Could you check a few things on this model? Use its own coordinates, in mm. Coordinates: 2 decimals unless noted, no trailing zeros. Loops run counter-clockwise (first coordinate to the right, second up) from the corner with the lowest first, then second, coordinate; pieces in that order, holes last. Notation, with made-up numbers: (-10.5, 88) - (30.5, 88) arc R25 cw to (30.5, 117) - close; hole circle Ø3 at (44.25, -32.75). An arc over 180 degrees is marked (long way). Use CSV: the item, a comma, the result in double quotes.
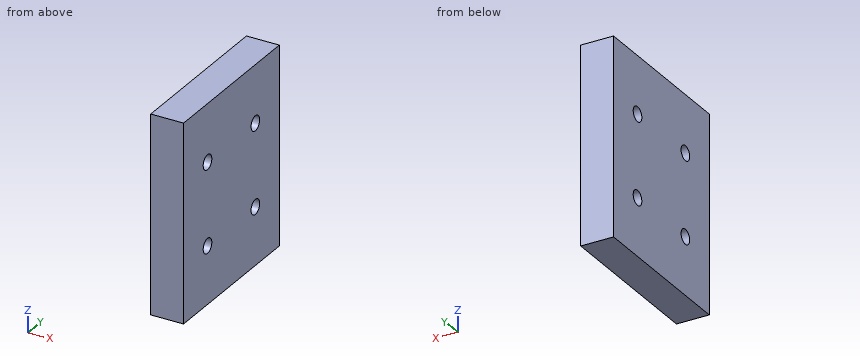
from build123d import *

# Parameters (mm, degrees)
SKETCH_1_W            = 120
SKETCH_1_H            = 100
EXTRUDE_1_DEPTH       = 20
HOLE_WIZARD_9_0_9_1_D = 9


with BuildPart() as part:
    # 草图1 → 凸台-拉伸1 (new body)
    with BuildSketch(Plane(origin=(0, 0, 0), x_dir=(0, 0, -1), z_dir=(1, 0, 0))):
        Rectangle(SKETCH_1_W, SKETCH_1_H)
    extrude(amount=EXTRUDE_1_DEPTH)

    # Ø9.0 (9) 直径孔1 (through all)
    with Locations(Plane(origin=(20, 0, 0), x_dir=(0, 0, -1), z_dir=(1, 0, 0))):
        with Locations((-25, 25), (25, 25), (-25, -25), (25, -25)):
            Hole(HOLE_WIZARD_9_0_9_1_D / 2)


solid = part.part
(1) Suppose I cut it at B-B (z = 25). Write out the boundary of the cut face in (x, y).
Computed:
outline,"(0, -50) - (20, -50) - (20, -29.5) - (0, -29.5) - close; (0, -20.5) - (20, -20.5) - (20, 20.5) - (0, 20.5) - close; (0, 29.5) - (20, 29.5) - (20, 50) - (0, 50) - close"
(2) Suppose I cut it at A-A (x = 11.25). Write out the boundary of the cut face in (y, z), plus the area to 3 significant figures.
Computed:
outline,"(-50, -60) - (50, -60) - (50, 60) - (-50, 60) - close; hole circle Ø9 at (-25, -25); hole circle Ø9 at (-25, 25); hole circle Ø9 at (25, -25); hole circle Ø9 at (25, 25)"
area,"11,700 mm²"
(3) Suppose I cut it at C-C (y = 25). Write out the boundary of the cut face in (x, z).
Computed:
outline,"(0, -60) - (20, -60) - (20, -29.5) - (0, -29.5) - close; (0, -20.5) - (20, -20.5) - (20, 20.5) - (0, 20.5) - close; (0, 29.5) - (20, 29.5) - (20, 60) - (0, 60) - close"
(4) Please list where these lines run through material, in increasing order: line 1 (Y direction, x = 8.25, z = 25); line 2 (Z direction, x = 8.5, y = 26.5).
Computed:
line 1,"y = -50 to -29.5, -20.5 to 20.5, 29.5 to 50"
line 2,"z = -60 to -29.24, -20.76 to 20.76, 29.24 to 60"
